CAD build for the part. Positions are in the model's coordinates, mm. A direction names the side the tool comes from. Coordinates: 2 decimals unless noted, no trailing zeros. Loops run counter-clockwise (first coordinate to the right, second up) from the corner with the lowest first, then second, coordinate; pieces in that order, holes last. Notation, with made-up numbers: (-39.5, 15.5) -> (-34.5, 15.5) arc R22 cw to (-34.5, 43.5) -> close; hole circle Ø1 at (34.5, 48.5). An arc over 180 degrees is marked (long way). Write each question's results on one line, items separated by ' | '.
```python
from build123d import *

# Parameters (mm, degrees)
SKETCH_2_R          = 20
CUT_EXTRUDE_1_DEPTH = 5
CUT_EXTRUDE_2_REACH = 424.606
SKETCH_3_R          = 11
SKETCH_5_R          = 120
SKETCH_5_R_2        = 80
CUT_EXTRUDE_3_DEPTH = 8
EXTRUDE_START       = 26
SKETCH_6_R          = 52.5
SKETCH_6_R_2        = 45
EXTRUDE_1_DEPTH     = 26
SKETCH_7_R          = 45
SKETCH_7_R_2        = 30
EXTRUDE_2_DEPTH     = 10
CHAMFER_1_SIZE      = 2
CHAMFER_2_SIZE      = 2


with BuildPart() as part:
    # 草图1 → 旋转1 (revolve)
    with BuildSketch(Plane.XY, mode=Mode.PRIVATE) as revolve_1_sk:
        with BuildLine():
            Line((60, 198.020625577), (132, 198.020625577))
            Line((132, 198.020625577), (135, 195.020625577))
            Line((135, 195.020625577), (135, 185.020625577))
            Line((135, 185.020625577), (200, 185.020625577))
            Line((200, 185.020625577), (200, 150.020625577))
            ThreePointArc((200, 150.020625577), (198.535533906, 146.485091671), (195, 145.020625577))
            Line((195, 145.020625577), (145, 145.020625577))
            Line((145, 145.020625577), (145, 140.020625577))
            Line((145, 140.020625577), (80, 140.020625577))
            Line((80, 140.020625577), (80, 87.020625577))
            Line((80, 87.020625577), (77, 84.020625577))
            Line((77, 84.020625577), (65, 84.020625577))
            Line((65, 84.020625577), (65, -72.979374423))
            Line((65, -72.979374423), (62, -75.979374423))
            Line((62, -75.979374423), (52.5, -75.979374423))
            Line((52.5, -75.979374423), (52.5, -131.979374423))
            Line((52.5, -131.979374423), (52.5, -133.979374423))
            Line((52.5, -133.979374423), (50.5, -133.979374423))
            Line((50.5, -133.979374423), (45, -133.979374423))
            Line((45, -133.979374423), (45, -167.979374423))
            Line((45, -167.979374423), (45, -168.979374423))
            Line((45, -168.979374423), (44, -168.979374423))
            Line((44, -168.979374423), (30, -168.979374423))
            Line((30, -168.979374423), (30, -36.979374423))
            Line((30, -36.979374423), (45, -20.479374423))
            Line((45, -20.479374423), (45, 177.020625577))
            Line((45, 177.020625577), (53, 193.020625577))
            Line((53, 193.020625577), (60, 193.020625577))
            Line((60, 193.020625577), (60, 198.020625577))
        make_face()
    revolve(revolve_1_sk.sketch.rotate(Axis((0, 246.142362889, 0), (0, -1, 0)), 90), axis=Axis((0, 246.142362889, 0), (0, -1, 0)))

    # 草图2 → 切除-拉伸1 (cut)
    with BuildSketch(Plane.XZ.offset(-145.020625577)):
        with Locations(Location((-120.208152802, 120.208152802, 0), (0, 0, 270))):
            Circle(SKETCH_2_R)
        with Locations(Location((-170, 0, 0), (0, 0, 270))):
            Circle(SKETCH_2_R)
        with Locations(Location((0, 170, 0), (0, 0, 270))):
            Circle(SKETCH_2_R)
        with Locations(Location((120.208152802, 120.208152802, 0), (0, 0, 270))):
            Circle(SKETCH_2_R)
        with Locations(Location((170, 0, 0), (0, 0, 270))):
            Circle(SKETCH_2_R)
        with Locations(Location((120.208152802, -120.208152802, 0), (0, 0, 270))):
            Circle(SKETCH_2_R)
        with Locations(Location((0, -170, 0), (0, 0, 270))):
            Circle(SKETCH_2_R)
        with Locations(Location((-120.208152802, -120.208152802, 0), (0, 0, 270))):
            Circle(SKETCH_2_R)
    extrude(amount=-CUT_EXTRUDE_1_DEPTH, mode=Mode.SUBTRACT)

    # 草图3 → 切除-拉伸2 (cut, up to next)
    with BuildSketch(Plane.XZ.offset(-145.020625577), mode=Mode.PRIVATE) as cut_extrude_2_sk1:
        with Locations(Location((-170, 0, 0), (0, 0, 270))):
            Circle(SKETCH_3_R)
    cut_extrude_2_tool1 = extrude(cut_extrude_2_sk1.sketch, amount=-CUT_EXTRUDE_2_REACH, mode=Mode.PRIVATE) & part.part
    # 草图3 → 切除-拉伸2 (cut, up to next)
    with BuildSketch(Plane.XZ.offset(-145.020625577), mode=Mode.PRIVATE) as cut_extrude_2_sk2:
        with Locations(Location((-120.208152802, 120.208152802, 0), (0, 0, 270))):
            Circle(SKETCH_3_R)
    cut_extrude_2_tool2 = extrude(cut_extrude_2_sk2.sketch, amount=-CUT_EXTRUDE_2_REACH, mode=Mode.PRIVATE) & part.part
    # 草图3 → 切除-拉伸2 (cut, up to next)
    with BuildSketch(Plane.XZ.offset(-145.020625577), mode=Mode.PRIVATE) as cut_extrude_2_sk3:
        with Locations(Location((0, 170, 0), (0, 0, 270))):
            Circle(SKETCH_3_R)
    cut_extrude_2_tool3 = extrude(cut_extrude_2_sk3.sketch, amount=-CUT_EXTRUDE_2_REACH, mode=Mode.PRIVATE) & part.part
    # 草图3 → 切除-拉伸2 (cut, up to next)
    with BuildSketch(Plane.XZ.offset(-145.020625577), mode=Mode.PRIVATE) as cut_extrude_2_sk4:
        with Locations(Location((120.208152802, 120.208152802, 0), (0, 0, 270))):
            Circle(SKETCH_3_R)
    cut_extrude_2_tool4 = extrude(cut_extrude_2_sk4.sketch, amount=-CUT_EXTRUDE_2_REACH, mode=Mode.PRIVATE) & part.part
    # 草图3 → 切除-拉伸2 (cut, up to next)
    with BuildSketch(Plane.XZ.offset(-145.020625577), mode=Mode.PRIVATE) as cut_extrude_2_sk5:
        with Locations(Location((170, 0, 0), (0, 0, 270))):
            Circle(SKETCH_3_R)
    cut_extrude_2_tool5 = extrude(cut_extrude_2_sk5.sketch, amount=-CUT_EXTRUDE_2_REACH, mode=Mode.PRIVATE) & part.part
    # 草图3 → 切除-拉伸2 (cut, up to next)
    with BuildSketch(Plane.XZ.offset(-145.020625577), mode=Mode.PRIVATE) as cut_extrude_2_sk6:
        with Locations(Location((120.208152802, -120.208152802, 0), (0, 0, 270))):
            Circle(SKETCH_3_R)
    cut_extrude_2_tool6 = extrude(cut_extrude_2_sk6.sketch, amount=-CUT_EXTRUDE_2_REACH, mode=Mode.PRIVATE) & part.part
    # 草图3 → 切除-拉伸2 (cut, up to next)
    with BuildSketch(Plane.XZ.offset(-145.020625577), mode=Mode.PRIVATE) as cut_extrude_2_sk7:
        with Locations(Location((0, -170, 0), (0, 0, 270))):
            Circle(SKETCH_3_R)
    cut_extrude_2_tool7 = extrude(cut_extrude_2_sk7.sketch, amount=-CUT_EXTRUDE_2_REACH, mode=Mode.PRIVATE) & part.part
    # 草图3 → 切除-拉伸2 (cut, up to next)
    with BuildSketch(Plane.XZ.offset(-145.020625577), mode=Mode.PRIVATE) as cut_extrude_2_sk8:
        with Locations(Location((-120.208152802, -120.208152802, 0), (0, 0, 270))):
            Circle(SKETCH_3_R)
    cut_extrude_2_tool8 = extrude(cut_extrude_2_sk8.sketch, amount=-CUT_EXTRUDE_2_REACH, mode=Mode.PRIVATE) & part.part
    add(cut_extrude_2_tool1.solids().sort_by_distance((-170, 145.020626, 0))[0], mode=Mode.SUBTRACT)
    add(cut_extrude_2_tool2.solids().sort_by_distance((-120.208153, 145.020626, 120.208153))[0], mode=Mode.SUBTRACT)
    add(cut_extrude_2_tool3.solids().sort_by_distance((0, 145.020626, 170))[0], mode=Mode.SUBTRACT)
    add(cut_extrude_2_tool4.solids().sort_by_distance((120.208153, 145.020626, 120.208153))[0], mode=Mode.SUBTRACT)
    add(cut_extrude_2_tool5.solids().sort_by_distance((170, 145.020626, 0))[0], mode=Mode.SUBTRACT)
    add(cut_extrude_2_tool6.solids().sort_by_distance((120.208153, 145.020626, -120.208153))[0], mode=Mode.SUBTRACT)
    add(cut_extrude_2_tool7.solids().sort_by_distance((0, 145.020626, -170))[0], mode=Mode.SUBTRACT)
    add(cut_extrude_2_tool8.solids().sort_by_distance((-120.208153, 145.020626, -120.208153))[0], mode=Mode.SUBTRACT)

    # 草图5 → 切除-拉伸3 (cut)
    with BuildSketch(Plane.XZ.offset(-140.020625577)):
        with Locations(Location((0, 0, 0), (0, 0, 270))):
            Circle(SKETCH_5_R)
        with Locations(Location((0, 0, 0), (0, 0, 90))):
            Circle(SKETCH_5_R_2, mode=Mode.SUBTRACT)
    extrude(amount=-CUT_EXTRUDE_3_DEPTH, mode=Mode.SUBTRACT)

    # 草图6 → 凸台-拉伸1 (add)
    with BuildSketch(Plane.XZ.offset(133.979374423).offset(EXTRUDE_START)):
        with Locations(Location((0, 0, 0), (0, 0, 90))):
            Circle(SKETCH_6_R)
        with Locations(Location((0, 0, 0), (0, 0, 90))):
            Circle(SKETCH_6_R_2, mode=Mode.SUBTRACT)
    extrude(amount=-EXTRUDE_1_DEPTH)

    # 草图7 → 凸台-拉伸2 (add)
    with BuildSketch(Plane.XZ.offset(168.979374423)):
        with Locations(Location((0, 0, 0), (0, 0, 90))):
            Circle(SKETCH_7_R)
        with Locations(Location((0, 0, 0), (0, 0, 90))):
            Circle(SKETCH_7_R_2, mode=Mode.SUBTRACT)
    extrude(amount=EXTRUDE_2_DEPTH)

    # 倒角1
    chamfer_1_edges = [part.edges().sort_by_distance(p)[0] for p in [
        (0, -159.979374423, -52.5),
    ]]
    chamfer(chamfer_1_edges, length=CHAMFER_1_SIZE)

    # 倒角2
    chamfer_2_edges = [part.edges().sort_by_distance(p)[0] for p in [
        (0, -178.979374423, -45),
    ]]
    chamfer(chamfer_2_edges, length=CHAMFER_2_SIZE)


solid = part.part
```
Q1. Pull direction X, two halves, no side cores. Call faces 1 (the flat face through (112, 150.021, -129)), 2 (the cylindrical face through (126.216, 147.486, -139.285)), 3 (the cylindrical face through (-15.77, -117.553, 50.076)), 4 (the flat face through (131, 185.021, -42)): +X half, -X half, draft (parallel to the pull), parting line (faces both ways), or undercut.
Results are:
face 1: undercut | face 2: undercut | face 3: parting line | face 4: draft
Q2. Drop flat-ended pins along their axis: pin 1 (13 mm diameter, centred on x = -120.21, z = 120.21, fed in from +Y); pin 2 (2 mm diameter, centred on y = -0.5, z = -17.5, fed in from +X); pin 3 (1.5 mm diameter, centred on x = -19.5, y = -69.5, fed in from +Z); pin 4 (1.5 mm diameter, centred on x = -41.5, z = 157.5, fed in from +Y). Give the stop position or say it passes through.
Results are:
pin 1: through | pin 2: x = 62.87 | pin 3: z = 62.24 | pin 4: y = 185.02
Q3. Cut at B-B on y = 26.5. Write the cut outline in (x, z), and give its area (3 significant figures).
Results are:
outline: circle Ø130 at (0, 0); hole circle Ø90 at (0, 0) | area: 6,910 mm^2
Q4. Wall check: L1, parallel to Z at x = -1.5, y = -46.5; L2, parallel to X at y = -67.5, z = 0; L3, parallel to X at y = 61.5, z = 0. Give the ranges that are in metal, low to high. Write a range as from..to.
Results are:
L1: -64.98..-29.96, 29.96..64.98 | L2: -65..-30, 30..65 | L3: -65..-45, 45..65
Q5. Cut at C-C on y = -92. Write the cut outline in (x, z), and give its area (3 significant figures).
Results are:
outline: circle Ø105 at (0, 0); hole circle Ø60 at (0, 0) | area: 5,830 mm^2
Q6. Cut at A-A on z = 0. Give the number of separate pieces and of enclosed holes in the cut face, and give its area (3 significant figures).
Results are:
separate pieces: 4 | enclosed holes: 0 | area: 28,900 mm^2
Q7. Which spindle directions (+Z, -Z, +X, -X, +Y, -Y) get a long thin tool onto all of the face, cutting with end or side? Do faces 5 (the cylindrical face through (0, 167, 181)), 6 (the cylindrical face through (39.923, 79.653, 20.765)), 7 (the cylindrical face through (189.83, 147.49, 2.6)). Say none if no direction does.
Results are:
face 5: +Y, -Y | face 6: +Y | face 7: -Y
